from build123d import *

# Parameters (mm, degrees)
STEPPED_BASE_BLOCK_DEPTH           = 61
STEPPED_BASE_BLOCK_DEPTH_BACK      = 5
BRACKET_PROFILE_SKETCH_R           = 25
BRACKET_PROFILE_SKETCH_R_2         = 12.5
BEARING_BOSS_DEPTH                 = 56
QUADRANT_MOUNTING_PLATE_DEPTH      = 12
QUADRANT_MOUNTING_PLATE_DEPTH_BACK = 5
SKETCH1_9_R                        = 6
UPRIGHT_WEB_DEPTH                  = 12
BASE_HOLES_SKETCH_R                = 8
BASE_THROUGH_HOLES_DEPTH           = 98


with BuildPart() as part:
    # Bracket Profile Sketch → Stepped Base Block (new, two sides: drawn at the far end of the back side and taken through both)
    with BuildSketch(Plane.XY.offset(-STEPPED_BASE_BLOCK_DEPTH_BACK)):
        with Locations((75, 36)):
            Circle(BRACKET_PROFILE_SKETCH_R)
        with Locations((75, 36)):
            Circle(BRACKET_PROFILE_SKETCH_R_2, mode=Mode.SUBTRACT)
    extrude(amount=STEPPED_BASE_BLOCK_DEPTH + STEPPED_BASE_BLOCK_DEPTH_BACK)

    # Sketch1_5 → Bearing Boss (add)
    with BuildSketch(Plane.XY):
        with BuildLine():
            Line((0, 16), (0, 0))
            Line((0, 0), (75, 0))
            Line((75, 0), (165, 0))
            Line((165, 0), (164.54886934, 27))
            ThreePointArc((164.54886934, 27), (149.458041876, 11.909172536), (134.367214412, 27))
            Line((134.367214412, 27), (134.3211598, 27))
            Line((134.3211598, 27), (98.323807579, 27))
            ThreePointArc((98.323807579, 27), (70.422620263, 11.422620263), (50, 36))
            Line((50, 36), (50, 16))
            Line((50, 16), (0, 16))
        make_face()
        with BuildLine():
            ThreePointArc((134.367214412, 27), (149.458041876, 11.909172536), (164.54886934, 27))
            Line((164.54886934, 27), (134.367214412, 27))
        make_face()
    extrude(amount=BEARING_BOSS_DEPTH)

    # Sketch1_9 → Quadrant Mounting Plate (add, two sides: drawn at the far end of the back side and taken through both)
    # profile 1 of 2: a face of its own
    with BuildSketch(Plane.XY.offset(-QUADRANT_MOUNTING_PLATE_DEPTH_BACK)):
        with BuildLine():
            Line((134.367214412, 27), (164.54886934, 27))
            ThreePointArc((164.54886934, 27), (141.745786384, 96.373835392), (75, 126))
            ThreePointArc((75, 126), (64.393398282, 121.606601718), (60, 111))
            ThreePointArc((60, 111), (64.393398282, 100.393398282), (75, 96))
            ThreePointArc((75, 96), (82.560257549, 95.521781776), (90, 94.094750193))
            ThreePointArc((90, 94.094750193), (124.13637209, 70.432788703), (134.725771353, 30.270057917))
            ThreePointArc((134.725771353, 30.270057917), (134.566433501, 28.8), (134.370917994, 27.334315001))
            ThreePointArc((134.370917994, 27.334315001), (134.368140336, 27.167167757), (134.367214412, 27))
        make_face()
        with Locations((150, 36)):
            Circle(SKETCH1_9_R, mode=Mode.SUBTRACT)
        with Locations((75, 111)):
            Circle(SKETCH1_9_R, mode=Mode.SUBTRACT)
        with Locations((139.951905284, 73.5)):
            Circle(SKETCH1_9_R, mode=Mode.SUBTRACT)
        with Locations((112.5, 100.951905284)):
            Circle(SKETCH1_9_R, mode=Mode.SUBTRACT)
    # profile 2 of 2: a face of its own
    with BuildSketch(Plane.XY.offset(-QUADRANT_MOUNTING_PLATE_DEPTH_BACK)):
        with BuildLine():
            ThreePointArc((134.367214412, 27), (149.458041876, 11.909172536), (164.54886934, 27))
            Line((164.54886934, 27), (134.367214412, 27))
        make_face()
    extrude(amount=QUADRANT_MOUNTING_PLATE_DEPTH + QUADRANT_MOUNTING_PLATE_DEPTH_BACK)

    # Sketch1_10 → Upright Web (add)
    with BuildSketch(Plane.XY):
        with BuildLine():
            Line((60, 61), (60, 56))
            ThreePointArc((60, 56), (75, 61), (90, 56))
            Line((90, 56), (90, 61))
            Line((90, 61), (90, 94.094750193))
            ThreePointArc((90, 94.094750193), (82.560257549, 95.521781776), (75, 96))
            ThreePointArc((75, 96), (64.393398282, 100.393398282), (60, 111))
            Line((60, 111), (60, 96))
            Line((60, 96), (60, 61))
        make_face()
    extrude(amount=UPRIGHT_WEB_DEPTH)

    # Base Holes Sketch → Base Through Holes (cut)
    with BuildSketch(Plane(origin=(0, 0, 0), x_dir=(1, 0, 0), z_dir=(0, 1, 0))):
        with Locations(Location((25, -31, 0), (0, 0, 90))):
            Circle(BASE_HOLES_SKETCH_R)
        with Locations(Location((139.54886934, -31, 0), (0, 0, 270))):
            Circle(BASE_HOLES_SKETCH_R)
    extrude(amount=BASE_THROUGH_HOLES_DEPTH, mode=Mode.SUBTRACT)


solid = part.part
For this review, take the finished solid that the model builds, in its own axes (mm). A direction names the side the tool comes from. Round coordinates to 2 decimals unless told otherwise and drop trailing zeros. Write each loop counter-clockwise with the first axis right and the second up, starting at its lowest first coordinate (ties: lowest second). Pieces come first, ordered by that corner, then holes. Notation, with made-up numbers: (21, -3) -> (62, -3) arc R21 ccw to (62, 8) -> close; hole circle Ø1 at (18, 9.25). An arc over 180 degrees is marked (long way). Put each result on its own line as item: value.
Q1. Consider section A-A on y = 92. State the section outline as (x, z) points.
Determined:
outline: (60, 0) -> (90, 0) -> (90, 12) -> (60, 12) -> close; (96.54, -5) -> (145.46, -5) -> (145.46, 12) -> (96.54, 12) -> close
Q2. Machinability: for faces 1 (the flat face through (81, 0, 28)), 2 (the flat face through (131.9, 27, 27.6)), 3 (the flat face through (81, 10, 0)), 4 (the flat face through (60, 84, 6)), 5 (the flat face through (63.5, 41.9, 61)), which of the approach directions +Z, -Z, +X, -X, +Y, -Y give a long, thin tool a straight path to every point of the face, cutting with its end or side? Answer none if there is none.
Determined:
face 1: +Z, -Z, +X, -X, -Y
face 2: +Z
face 3: -Z, -Y
face 4: +Z, -Z, -X, +Y
face 5: +Z, +X, -X, +Y, -Y
Q3. Consider section D-D on z = 42. State the section outline as (x, y) points, and give its area (3 significant figures).
Determined:
outline: (0, 0) -> (165, 0) -> (164.55, 27) -> (98.32, 27) arc R25 ccw (long way) to (50, 36) -> (50, 16) -> (0, 16) -> close; hole circle Ø25 at (75, 36)
area: 4,830 mm^2
Q4. Consider section C-C on x = 150. State the section outline as (y, z) points, and give its area (3 significant figures).
Determined:
outline: (0, 0) -> (11.92, 0) -> (11.92, -5) -> (30, -5) -> (30, 12) -> (27, 12) -> (27, 56) -> (0, 56) -> close; (42, -5) -> (85.75, -5) -> (85.75, 12) -> (42, 12) -> close
area: 2,380 mm^2
Q5. The part is to be moulded in two halves that separate along X. For faces 6 (the flat face through (50, 26, 28)), 7 (the cylindrical face through (145.24, 32.35, 3.38)), 8 (the flat face through (90, 75, 6)), 9 (the flat face through (112, 88, 12)), say which applies: released by +X, released by -X, zero draft, split by the parting line, or undercut.
Determined:
face 6: released by -X
face 7: undercut
face 8: undercut
face 9: zero draft
Q6. Consider section B-B on z = 30.5. State the section outline as (x, y) points.
Determined:
outline: (0, 0) -> (17.02, 0) -> (17.02, 16) -> (0, 16) -> close; (32.98, 0) -> (131.56, 0) -> (131.56, 27) -> (98.32, 27) arc R25 ccw (long way) to (50, 36) -> (50, 16) -> (32.98, 16) -> close; (147.53, 0) -> (165, 0) -> (164.55, 27) -> (147.53, 27) -> close; hole circle Ø25 at (75, 36)
Q7. Clearance check with flat-ended pins moving along their axes: pin 1 Ø12 at (x, z) = (67.5, 35) entering from +Y; pin 2 Ø8 at (y, z) = (36, 26) entering from -X; pin 3 Ø9.5 at (y, z) = (90, 7) entering from -X. State where each tip first meets the part, or that it passes through.
Determined:
pin 1: stops at y = 60.95
pin 2: stops at x = 50
pin 3: stops at x = 60
Q8. To check wall thickness, follow L1, parallel to Y at x = 75, z = 2; L2, parallel to X at y = 13, z = 31; L3, parallel to Y at x = 112.5, z = 6. State the ranges of each line that lie inside material, in increasing order. Write a range as [from, to].
Determined:
L1: y = [0, 23.5], [48.5, 105], [117, 126]
L2: x = [0, 17], [33, 131.55], [147.55, 164.78]
L3: y = [0, 27], [82.84, 94.95], [106.95, 117.82]
